Geometry check sheet. Reference: the model listing, model coordinates, mm. Round coordinates to 2 decimals unless told otherwise and drop trailing zeros. Write each loop counter-clockwise with the first axis right and the second up, starting at its lowest first coordinate (ties: lowest second). Pieces come first, ordered by that corner, then holes. Notation, with made-up numbers: (11.5, 18) - (56.5, 18) arc R19 cw to (56.5, 54) - close; hole circle Ø11 at (33.5, 20). An arc over 180 degrees is marked (long way). Return JSON: item names as keys, results as strings.
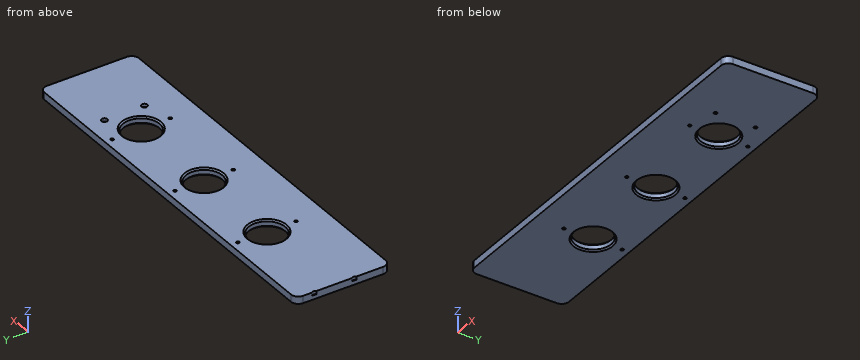
```python
from build123d import *

# Parameters (mm, degrees)
SKETCH_1_W                   = 530
SKETCH_1_H                   = 130
EXTRUDE_1_DEPTH              = 10
HOLE_WIZARD_M4_1_D           = 4.5
HOLE_WIZARD_M4_1_CBORE_D     = 8
HOLE_WIZARD_M4_1_CBORE_DEPTH = 4.4
PATTERN_LINEAR_1_COUNT       = 2
PATTERN_LINEAR_1_PITCH       = 436
SKETCH_14_R                  = 25
CUT_EXTRUDE_1_DEPTH          = 274.03845883
CHAMFER_1_SIZE               = 2
HOLE_WIZARD_M5_2_D           = 4.2
FILLET_1_R                   = 10


with BuildPart() as part:
    # 草图1 → 凸台-拉伸1 (new body)
    with BuildSketch(Plane.XY):
        Rectangle(SKETCH_1_W, SKETCH_1_H)
    extrude(amount=EXTRUDE_1_DEPTH)

    # M4 六角凹头螺钉的柱形沉头孔1 (through all)
    with Locations(Plane(origin=(0, 0, 10), x_dir=(-1, 0, 0), z_dir=(0, 0, 1))):
        with Locations((-168.5, 15), (-168.5, -40)):
            hole_wizard_m4_1 = CounterBoreHole(HOLE_WIZARD_M4_1_D / 2, HOLE_WIZARD_M4_1_CBORE_D / 2, HOLE_WIZARD_M4_1_CBORE_DEPTH)

    # 阵列(线性)1: M4 六角凹头螺钉的柱形沉头孔1 ×2
    with Locations(*[(-i * PATTERN_LINEAR_1_PITCH, 0, 0) for i in range(1, PATTERN_LINEAR_1_COUNT)]):
        add(hole_wizard_m4_1, mode=Mode.SUBTRACT)

    # 草图14 → 切除-拉伸1 (cut, through all)
    with BuildSketch(Plane.XY.offset(10)):
        with Locations((-130, 15)):
            Circle(SKETCH_14_R)
        with Locations((0, 15)):
            Circle(SKETCH_14_R)
        with Locations((130, 15)):
            Circle(SKETCH_14_R)
    extrude(amount=-CUT_EXTRUDE_1_DEPTH, mode=Mode.SUBTRACT)

    # 倒角1
    chamfer_1_edges = [part.edges().sort_by_distance(p)[0] for p in [
        (-155, 15, 0),
        (-155, 15, 10),
        (-25, 15, 0),
        (-25, 15, 10),
        (105, 15, 0),
        (105, 15, 10),
    ]]
    chamfer(chamfer_1_edges, length=CHAMFER_1_SIZE)

    # M5 螺纹孔2 (through all)
    with Locations(Plane.XY.offset(10)):
        with Locations((130, 55), (-130, -25), (-130, 55), (0, 55), (0, -25), (130, -25)):
            Hole(HOLE_WIZARD_M5_2_D / 2)

    # 圆角1
    fillet_1_edges = [part.edges().sort_by_distance(p)[0] for p in [
        (265, -65, 5),
        (-265, -65, 5),
        (-265, 65, 5),
        (265, 65, 5),
    ]]
    fillet(fillet_1_edges, radius=FILLET_1_R)


solid = part.part
```
(1) Section check B-B, the plane z = 4. Give the number of separate pieces and of enclosed holes in the cut face, plus the area to 3 significant figures.
Response values:
{"separate pieces": "1", "enclosed holes": "11", "area": "62,800 mm^2"}
(2) Section check A-A, the plane y = 15. Enter the section's corners in (x, z).
Response values:
{"outline": "(-265, 0) - (-157, 0) - (-155, 2) - (-155, 8) - (-157, 10) - (-265, 10) - close; (-105, 2) - (-103, 0) - (-27, 0) - (-25, 2) - (-25, 8) - (-27, 10) - (-103, 10) - (-105, 8) - close; (25, 2) - (27, 0) - (103, 0) - (105, 2) - (105, 8) - (103, 10) - (27, 10) - (25, 8) - close; (155, 2) - (157, 0) - (265, 0) - (265, 10) - (157, 10) - (155, 8) - close"}
(3) Material ranges on line 1 along Y through (x, z) = (130, 5); line 2 along Y through (x, z) = (168.5, 4.05); line 3 along X through (y, z) = (54.5, 8), recorded low to high. Write a range as [from, to].
Response values:
{"line 1": "y = [-65, -27.1], [-22.9, -10], [40, 52.9], [57.1, 65]", "line 2": "y = [-65, -17.25], [-12.75, 37.75], [42.25, 65]", "line 3": "x = [-265, -132.04], [-127.96, -2.04], [2.04, 127.96], [132.04, 265]"}
(4) Gauge pin test, flat ends, axial feed: pin 1 (3.5 mm diameter, centred on x = 130, y = 55, fed in from -Z); pin 2 (9 mm diameter, centred on x = 168.5, y = -15, fed in from -Z); pin 3 (2.5 mm diameter, centred on x = 167, y = -15, fed in from +Z). Record the tip position at first contact, or that the pin passes through.
Response values:
{"pin 1": "passes through", "pin 2": "stops at z = 0", "pin 3": "stops at z = 5.6"}
